Here's how the part is built. I have some questions about the finished solid (model axes, mm). A direction names the side the tool comes from. Round coordinates to 2 decimals unless told otherwise and drop trailing zeros. Order: outer loops, then holes, each group sorted by start corner. A loop starts at its lowest first (then second) coordinate and runs counter-clockwise, first axis right, second up. Notation, with made-up numbers: M -13.75,-34 L 27.25,-34 A20 ccw 27.25,-20 Z; hole C 68.25,73.5 d3. An arc over 180 degrees is marked long. Use one line per item in the form item = value. Start each with the question number.
```python
from build123d import *
from OCP.BRepFilletAPI import BRepFilletAPI_MakeChamfer

# Parameters (mm, degrees)
BOSS_EXTRUDE1_DEPTH                          = 9
SKETCH2_W                                    = 70
SKETCH2_H                                    = 3
SKETCH2_W_2                                  = 10
SKETCH2_H_2                                  = 4
BOSS_EXTRUDE2_DEPTH                          = 6
CBORE_FOR_M5_SLOTTED_CHEESE_HEAD_SCR_2_COUNT = 2
CBORE_FOR_M5_SLOTTED_CHEESE_HEAD_SCR_2_PITCH = 50
SKETCH13_R                                   = 1.5
CUT_EXTRUDE1_DEPTH                           = 75.873226189
CHAMFER3_SIZE                                = 0.5
CHAMFER3_SIZE2                               = 0.288675135
CHAMFER9_SIZE                                = 2
FILLET1_R                                    = 1
CHAMFER6_SIZE                                = 0.5
CHAMFER7_SIZE                                = 0.5
CUT_EXTRUDE2_DEPTH                           = 75.873226189
CHAMFER8_SIZE                                = 0.5


with BuildPart() as part:
    # Sketch1 → Boss-Extrude1 (new body)
    with BuildSketch(Plane(origin=(0, 0, 0), x_dir=(1, 0, 0), z_dir=(0, 1, 0))):
        Polygon((10, 21), (60, 21), (60, 25), (70, 25), (70, 0), (0, 0), (0, 25), (10, 25), align=None)
    extrude(amount=BOSS_EXTRUDE1_DEPTH)

    # Sketch2 → Boss-Extrude2 (add)
    with BuildSketch(Plane(origin=(0, 9, 0), x_dir=(1, 0, 0), z_dir=(0, 1, 0))):
        with Locations((35, 16.5)):
            Rectangle(SKETCH2_W, SKETCH2_H)
        with Locations((65, 23)):
            Rectangle(SKETCH2_W_2, SKETCH2_H_2)
        with Locations((5, 23)):
            Rectangle(SKETCH2_W_2, SKETCH2_H_2)
    extrude(amount=BOSS_EXTRUDE2_DEPTH)

    # Sketch12 → CBORE for M5 Slotted cheese head screws1 (revolve, cut)
    with BuildSketch(Plane(origin=(10, 9, -7.5), x_dir=(0, 0, 1), z_dir=(1, 0, 0))):
        Polygon((0, 0), (0, 9), (2.75, 9), (2.75, 6), (5, 6), (5, 0.025), (5.025, 0), align=None)
    cbore_for_m5_slotted_cheese_head_screws1 = revolve(axis=Axis((10, 15.35, -7.5), (0, -1, 0)), mode=Mode.SUBTRACT)

    # CBORE for M5 Slotted cheese head scr 2: CBORE for M5 Slotted cheese head screws1 ×2
    with Locations(*[(i * CBORE_FOR_M5_SLOTTED_CHEESE_HEAD_SCR_2_PITCH, 0, 0) for i in range(1, CBORE_FOR_M5_SLOTTED_CHEESE_HEAD_SCR_2_COUNT)]):
        add(cbore_for_m5_slotted_cheese_head_screws1, mode=Mode.SUBTRACT)

    # Sketch13 → Cut-Extrude1 (cut, through all)
    with BuildSketch(Plane(origin=(0, 9, 0), x_dir=(1, 0, 0), z_dir=(0, 1, 0))):
        with Locations(Location((45.000000243, 7.502702464, 0), (0, 0, 270))):
            Circle(SKETCH13_R)
        with Locations(Location((25.000000243, 7.502702464, 0), (0, 0, 270))):
            Circle(SKETCH13_R)
    extrude(amount=-CUT_EXTRUDE1_DEPTH, mode=Mode.SUBTRACT)

    # Chamfer3: one chamfer whose edges measure the first distance from different faces: ONE call of the kernel's chamfer builder (chamfer() names one face for all edges)
    chamfer3_edges_1 = [part.edges().sort_by_distance(p)[0] for p in [
        (5, 15, -21),
    ]]
    chamfer3_side_1 = [part.faces().sort_by_distance(p)[0] for p in [
        (5, 12, -21),
    ]]
    chamfer3_edges_2 = [part.edges().sort_by_distance(p)[0] for p in [
        (65, 15, -21),
    ]]
    chamfer3_side_2 = [part.faces().sort_by_distance(p)[0] for p in [
        (65, 12, -21),
    ]]
    chamfer3 = BRepFilletAPI_MakeChamfer(part.part.solid().wrapped)
    for e in chamfer3_edges_1:
        chamfer3.Add(CHAMFER3_SIZE, CHAMFER3_SIZE2, e.wrapped, chamfer3_side_1[0].wrapped)  # the first distance lies on this face
    for e in chamfer3_edges_2:
        chamfer3.Add(CHAMFER3_SIZE, CHAMFER3_SIZE2, e.wrapped, chamfer3_side_2[0].wrapped)  # the first distance lies on this face
    add(Compound.cast(chamfer3.Shape()), mode=Mode.REPLACE)

    # Chamfer9
    chamfer9_edges = [part.edges().sort_by_distance(p)[0] for p in [
        (35, 9, -21),
    ]]
    chamfer(chamfer9_edges, length=CHAMFER9_SIZE)

    # Fillet1
    fillet1_edges = [part.edges().sort_by_distance(p)[0] for p in [
        (10, 3.5, -21),
        (60, 3.5, -21),
    ]]
    fillet(fillet1_edges, radius=FILLET1_R)

    # Chamfer6
    chamfer6_edges = [part.edges().sort_by_distance(p)[0] for p in [
        (65, 0, -25),
        (70, 0, -12.5),
        (35, 0, 0),
        (0, 0, -12.5),
        (70, 9, -7.5),
        (0, 7.5, -25),
        (10, 7.5, -25),
        (60, 7.5, -25),
        (70, 7.5, -25),
        (70, 4.5, 0),
        (0, 4.5, 0),
        (0, 9, -7.5),
        (70, 9, -19.5),
        (0, 12, -18),
        (0, 12, -15),
        (70, 12, -15),
        (70, 12, -18),
        (0, 15, -16.5),
        (35, 15, -15),
        (70, 15, -16.5),
        (0, 9, -19.5),
        (0, 15, -23.144337567),
        (5, 15, -25),
        (65, 15, -25),
        (5, 0, -25),
        (70, 15, -23.144337567),
        (35, 9, 0),
        (70, 11.75, -21),
        (70, 14.75, -21.144337567),
        (0, 11.75, -21),
        (0, 14.75, -21.144337567),
    ]]
    chamfer(chamfer6_edges, length=CHAMFER6_SIZE)

    # Chamfer7
    chamfer7_edges = [part.edges().sort_by_distance(p)[0] for p in [
        (25.000000243, 0, -9.002702464),
        (25.000000243, 9, -9.002702464),
    ]]
    chamfer(chamfer7_edges, length=CHAMFER7_SIZE)

    # Sketch14 → Cut-Extrude2 (cut, through all)
    with BuildSketch(Plane(origin=(0, 9, 0), x_dir=(1, 0, 0), z_dir=(0, 1, 0))):
        with BuildLine():
            Line((43.500000243, 9.002702464), (46.500000243, 9.002702464))
            ThreePointArc((46.500000243, 9.002702464), (48.000000243, 7.502702464), (46.500000243, 6.002702464))
            Line((46.500000243, 6.002702464), (43.500000243, 6.002702464))
            ThreePointArc((43.500000243, 6.002702464), (42.000000243, 7.502702464), (43.500000243, 9.002702464))
        make_face()
    extrude(amount=-CUT_EXTRUDE2_DEPTH, mode=Mode.SUBTRACT)

    # Chamfer8
    chamfer8_edges = [part.edges().sort_by_distance(p)[0] for p in [
        (45.000000243, 0, -9.002702464),
        (45.000000243, 0, -6.002702464),
        (45.000000243, 9, -6.002702464),
        (45.000000243, 9, -9.002702464),
        (42.000000243, 9, -7.502702464),
        (48.000000243, 9, -7.502702464),
        (42.000000243, 0, -7.502702464),
        (48.000000243, 0, -7.502702464),
    ]]
    chamfer(chamfer8_edges, length=CHAMFER8_SIZE)


solid = part.part
```
1) If we mould it in two halves opening along Z, with no side actions, what happens to faces 1 (the flat face through (35, 4, 0)), 2 (the flat face through (35, 15, -17)), 3 (the flat face through (5, 12, -21))? For each: +Z half, -Z half, draft (parallel to the pull), parting line (faces both ways), or undercut.
2) On a 3-axis mill with a long thin cutter (end or side, diameter ignored), from which of +Z, -Z, +X, -X, +Y, -Y can I reach the whole of each face in a straight line? I mean faces 4 (the flat face through (45, 5, -6.003)), 5 (the conical face through (48.135, 0.365, -7.467)), 6 (the flat face through (62, 3, -10)). Say none if no direction works.
3) If we section it at C-C on x = 17.5: Write out the boundary of the cut face in (y, z), then the cut area to 3 significant figures.
4) Will these pins go through, and if not, where does the flat tip stop? pin 1 Ø8 at (x, z) = (60, -7) entering from +Y; pin 2 Ø6.5 at (x, y) = (33, 11) entering from -Z; pin 3 Ø11.5 at (x, z) = (33, -8) entering from +Y.
5) If I drill on line 1 (X direction, y = 7.6, z = -7.5); line 2 (Y direction, x = 61.5, z = -13.25); line 3 (X direction, y = 2.75, z = -5.5), over which ranges is the centre line in solid material (lowest first)?
6) If we section it at A-A on x = 25: Write out the boundary of the cut face in (y, z), then the cut area to 3 significant figures.
7) If we section it at D-D on z = -13.5: Write out the boundary of the cut face in (x, y).
8) If we section it at B-B on y = 13: Write out the boundary of the cut face in (x, z), then the cut area to 3 significant figures.
Completed:
q1.face_1 = +Z half
q1.face_2 = draft
q1.face_3 = undercut
q2.face_4 = +Y, -Y
q2.face_5 = -Y
q2.face_6 = +Y
q3.outline = M 0,-21 L 7,-21 L 9,-19 L 9,-18 L 15,-18 L 15,-15.5 L 14.5,-15 L 9,-15 L 9,-0.5 L 8.5,0 L 0.5,0 L 0,-0.5 Z
q3.area = 205 mm²
q4.pin_1 = 3
q4.pin_2 = -20.25
q4.pin_3 = 9
q5.line_1 = 0 to 5, 15 to 23.5, 26.5 to 42, 48 to 55, 65 to 70
q5.line_2 = 0 to 9
q5.line_3 = 0 to 8.11, 11.89 to 58.11, 61.89 to 70
q6.outline = M 0,-21 L 7,-21 L 9,-19 L 9,-18 L 15,-18 L 15,-15.5 L 14.5,-15 L 9,-15 L 9,-9.5 L 8.5,-9 L 0.5,-9 L 0,-9.5 Z; M 0,-5.5 L 0.5,-6 L 8.5,-6 L 9,-5.5 L 9,-0.5 L 8.5,0 L 0.5,0 L 0,-0.5 Z
q6.area = 177 mm²
q7.outline = M 0,0.5 L 0.5,0 L 69.5,0 L 70,0.5 L 70,8.5 L 69.5,9 L 0.5,9 L 0,8.5 Z
q8.outline = M 0,-24.5 L 0.5,-25 L 9.5,-25 L 10,-24.5 L 10,-21 L 0.5,-21 L 0,-21.5 Z; M 0,-17.5 L 0.5,-18 L 69.5,-18 L 70,-17.5 L 70,-15.5 L 69.5,-15 L 0.5,-15 L 0,-15.5 Z; M 60,-24.5 L 60.5,-25 L 69.5,-25 L 70,-24.5 L 70,-21.5 L 69.5,-21 L 60,-21 Z
q8.area = 289 mm²
